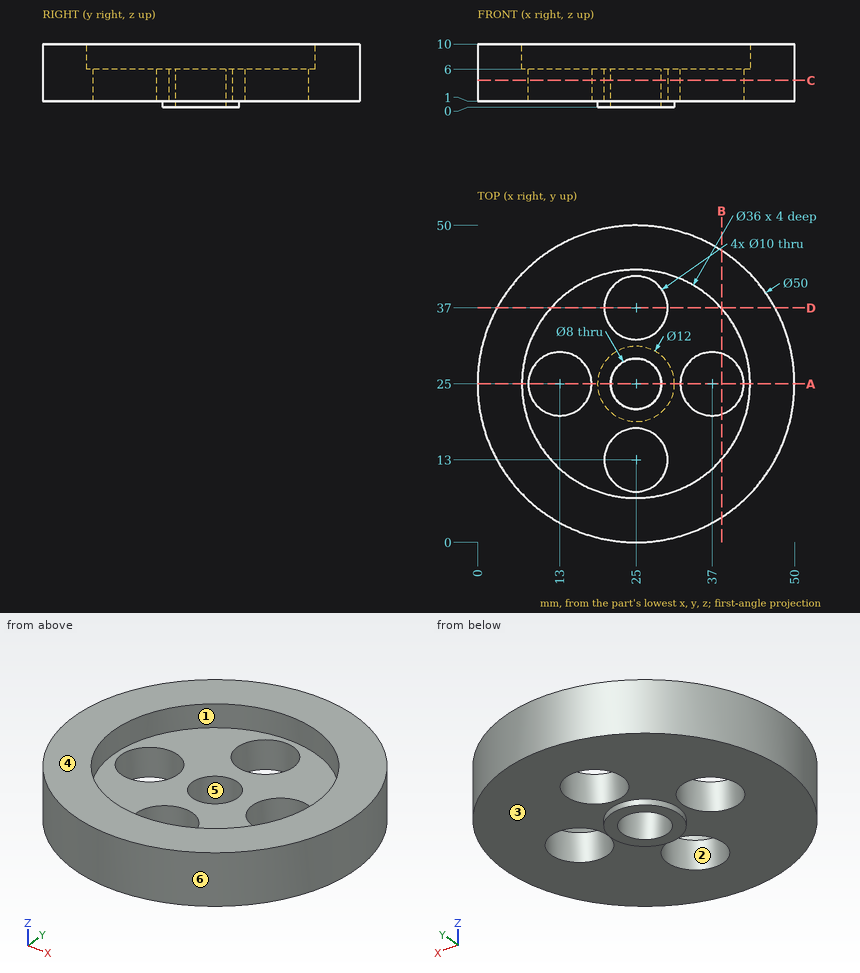
Geometry check sheet. Reference: drawing and pictorial views, mm from the part's lowest x, y, z. A direction names the side the tool comes from. Give positions to 0.01 mm unless a question says otherwise; leave off trailing zeros. Write each loop counter-clockwise with the first axis right and the second up, starting at its lowest first coordinate (ties: lowest second). Pieces come first, ordered by that corner, then holes. Notation, with made-up numbers: (25, -28.75) -> (82, -28.75) arc R34 cw to (82, 9.25) -> close; hole circle Ø9 at (16, 2.25). An arc over 180 degrees is marked (long way). One line per question, with ' | ' between items.
Item 1: Depth check by flat-ended pin: pin 1 (2 mm diameter, centred on x = 6, z = 6, fed in from +Y); pin 2 (3 mm diameter, centred on y = 44.5, z = 5.5, fed in from -X); pin 3 (4 mm diameter, centred on x = 41.5, z = 5, fed in from -Y). Enter the tip coordinate at first touch or a pass-through.
Determined:
pin 1: y = 42.35 | pin 2: x = 7.65 | pin 3: y = 4.63
Item 2: Sectioned sample at C-C, the plane z = 4.25. Record the boundary of the cut face in (x, y), plus the area to 3 significant figures.
Determined:
outline: circle Ø50 at (25, 25); hole circle Ø10 at (13, 25); hole circle Ø10 at (25, 13); hole circle Ø10 at (25, 37); hole circle Ø8 at (25, 25); hole circle Ø10 at (37, 25) | area: 1,600 mm^2
Item 3: Sectioned sample at A-A, the plane y = 25. Record the boundary of the cut face in (x, z), plus the area to 3 significant figures.
Determined:
outline: (0, 1) -> (8, 1) -> (8, 6) -> (7, 6) -> (7, 10) -> (0, 10) -> close; (18, 1) -> (19, 1) -> (19, 0) -> (21, 0) -> (21, 6) -> (18, 6) -> close; (29, 0) -> (31, 0) -> (31, 1) -> (32, 1) -> (32, 6) -> (29, 6) -> close; (42, 1) -> (50, 1) -> (50, 10) -> (43, 10) -> (43, 6) -> (42, 6) -> close | area: 170 mm^2
Item 4: Sectioned sample at D-D, the plane y = 37. Record the boundary of the cut face in (x, z).
Determined:
outline: (3.07, 1) -> (20, 1) -> (20, 6) -> (11.58, 6) -> (11.58, 10) -> (3.07, 10) -> close; (30, 1) -> (46.93, 1) -> (46.93, 10) -> (38.42, 10) -> (38.42, 6) -> (30, 6) -> close
Item 5: Draft check along X on the marked faces 4, 5 and 6. Enter one of: released by +X, released by -X, zero draft, split by the parting line, or undercut.
Determined:
face 4: zero draft | face 5: undercut | face 6: split by the parting line
Item 6: Scan lines: line 1 along Y through (x, z) = (25, 2.15); line 2 along Y through (x, z) = (25, 8.95); line 3 along Y through (x, z) = (20.5, 1.75). Record each from-to range of solid material in increasing order.
Determined:
line 1: 0 to 8, 18 to 21, 29 to 32, 42 to 50 | line 2: 0 to 7, 43 to 50 | line 3: 0.41 to 10.82, 15.18 to 34.82, 39.18 to 49.59
Item 7: Sectioned sample at B-B, the plane x = 38.5. Record the boundary of the cut face in (y, z).
Determined:
outline: (3.96, 1) -> (20.23, 1) -> (20.23, 6) -> (13.09, 6) -> (13.09, 10) -> (3.96, 10) -> close; (29.77, 1) -> (46.04, 1) -> (46.04, 10) -> (36.91, 10) -> (36.91, 6) -> (29.77, 6) -> close
Item 8: Access from +Z, -Z, +X, -X, +Y, -Y to the whole of each face (thin tool, end or side, straight path). Record for the marked faces 1, 2 and 3.
Determined:
face 1: +Z | face 2: +Z, -Z | face 3: -Z
